from build123d import *

# Parameters (mm, degrees)
FILLET_1_R          = 0.5
CHAMFER_1_SIZE      = 2.598076211
CHAMFER_1_SIZE2     = 1.5
SKETCH_2_R          = 1.69
CUT_EXTRUDE_1_DEPTH = 500


with BuildPart() as part:
    # 草图1 → Revolve 730 (revolve)
    with BuildSketch(Plane.XY, mode=Mode.PRIVATE) as revolve_730_sk:
        with BuildLine():
            Line((0, 0), (34.5, 0))
            Line((34.5, 0), (34.5, 5))
            Line((34.5, 5), (2.5, 5))
            Line((2.5, 5), (2.5, 5.75))
            ThreePointArc((2.5, 5.75), (1.25, 7), (0, 5.75))
            Line((0, 5.75), (0, 0))
        make_face()
    revolve(revolve_730_sk.sketch.rotate(Axis((0, 0, 0), (1, 0, 0)), 90), axis=Axis((0, 0, 0), (1, 0, 0)))

    # 圆角1
    fillet_1_edges = [part.edges().sort_by_distance(p)[0] for p in [
        (2.5, 0, -5),
    ]]
    fillet(fillet_1_edges, radius=FILLET_1_R)

    # 倒角1
    chamfer_1_edges = [part.edges().sort_by_distance(p)[0] for p in [
        (34.5, 0, -5),
    ]]
    chamfer_1_side = [part.faces().sort_by_distance(p)[0] for p in [
        (18.75, 0, -5),
    ]]
    chamfer(chamfer_1_edges, length=CHAMFER_1_SIZE, length2=CHAMFER_1_SIZE2, reference=chamfer_1_side[0])

    # 草图2 → 切除-拉伸1 (cut, symmetric)
    with BuildSketch(Plane(origin=(0, 0, 0), x_dir=(1, 0, 0), z_dir=(0, 1, 0))):
        with Locations(Location((30.5, 0, 0), (0, 0, 326.051586003))):
            Circle(SKETCH_2_R)
    extrude(amount=CUT_EXTRUDE_1_DEPTH, both=True, mode=Mode.SUBTRACT)


solid = part.part
Input: part model. Units: mm. Frame: model coordinates. Give positions to 0.01 mm unless a question says otherwise; leave off trailing zeros. Loops run counter-clockwise (first coordinate to the right, second up) from the corner with the lowest first, then second, coordinate; pieces in that order, holes last. Notation, with made-up numbers: M -26,54 L -12,54 A23 ccw -12,66 Z; hole C -24,86.5 d9. An arc over 180 degrees is marked long. Use CSV: the item, a comma, the result in double quotes.
(1) Pin query (flat end, axial travel): P1, Ø8, axis at y = 1.5, z = 3.5, coming from the +X side; P2, Ø4, axis at x = 22.5, z = -4.5, coming from the -Y side; P3, Ø1.5, axis at x = 16, y = -0.5, coming from the +Z side; P4, Ø1, axis at x = 28.5, y = 2, coming from the +Z side. Return the tip coordinate at first contact, or that it passes through.
Outcome:
P1,"stops at x = 34.5"
P2,"stops at y = -4.33"
P3,"stops at z = 5"
P4,"stops at z = 4.77"
(2) Section D-D, the plane x = 7. Return loops of the section in (y, z).
Outcome:
outline,"C 0,0 d10"
(3) Section A-A, the plane z = 0. Return loops of the section in (x, y), plus the area to 3 significant figures.
Outcome:
outline,"M 0,-5.75 A1.25 ccw 2.5,-5.75 L 2.5,-5.5 A0.5 cw 3,-5 L 28.81,-5 L 28.81,5 L 3,5 A0.5 cw 2.5,5.5 L 2.5,5.75 A1.25 ccw 0,5.75 Z; M 32.19,-4.83 L 34.5,-3.5 L 34.5,3.5 L 32.19,4.83 Z"
area,"316 mm²"
(4) Section C-C, the plane x = 2. Return loops of the section in (y, z), plus the area to 3 significant figures.
Outcome:
outline,"C 0,0 d13.5"
area,"143 mm²"
(5) Material intervals for L1, parallel to X at y = 0, z = 0; L2, parallel to X at y = 2.75, z = 0.5; L3, parallel to Y at x = 24.5, z = 0, sorted ascending. Write a range as [from, to].
Outcome:
L1,"x = [0, 28.81], [32.19, 34.5]"
L2,"x = [0, 28.89], [32.11, 34.5]"
L3,"y = [-5, 5]"
(6) Section B-B, the plane x = 30.5. Return loops of the section in (y, z).
Outcome:
outline,"M -4.71,-1.69 A5 ccw 4.71,-1.69 Z; M -4.71,1.69 L 4.71,1.69 A5 ccw Z"
(7) Pull-direction query (Z, two-part tool) for faces 1 (the face through (17.25, -1.5, 4.77)), 2 (the face through (28.813, 0.07, 0.104)), 3 (the face through (34.5, 0, 0)); classes: pulls with the +Z half, pulls with the -Z half, needs draft (parallel to the pull), parting line crosses it, or undercut.
Outcome:
face 1,"parting line crosses it"
face 2,"undercut"
face 3,"needs draft"
